Answer from the drawing. Dimensions are ordinates in mm from the lowest x, y and z of the part. A direction names the side the tool comes from. Coordinates: 2 decimals unless noted, no trailing zeros. Write each loop counter-clockwise with the first axis right and the second up, starting at its lowest first coordinate (ties: lowest second). Pieces come first, ordered by that corner, then holes. Notation, with made-up numbers: (46.25, 43.25) -> (86.25, 43.25) arc R18 cw to (86.25, 47.25) -> close; hole circle Ø9 at (59.25, 38). An arc over 180 degrees is marked (long way). One line per item, written item: value. Start each with the question number.
1. Find section C-C, the plane y = 10. Write down the section's boundary in (x, z), and give its area (3 significant figures).
2. For the marked faces 5 and 6, determine the directions among +Z, -Z, +X, -X, +Y, -Y from which every point of the face is accessible in a straight line to the end or side of a thin tool.
3. For a pull along X with two mould halves and no side action, classify the marked faces 1, 2, 3 and 4 as pulls with the +X half, pulls with the -X half, needs draft (parallel to the pull), parting line crosses it, or undercut.
4. Find section B-B, the plane x = 50. Write down the section's boundary in (y, z).
5. Given P1, Ø11, axis at x = 47.5, y = 7.5, coming from the -Z side; P2, Ø6.5, axis at x = 50, y = 10, coming from the -Z side, each flat-ended and moving along its own axis, determine where each tip first touches the part or whether it passes through.
6. Find section A-A, the plane z = 1.25. Write down the section's boundary in (x, y).
7. Find section D-D, the plane z = 10.25. Write down the section's boundary in (x, y), and give its area (3 significant figures).
8. Consider line 1 along Y through (x, z) = (50, 4.4); line 2 along Y through (x, z) = (50, 8); line 3 along X through (y, z) = (25.5, 7.25) (1 decimal). Determine where each line is inside the solid, lowest interval first.
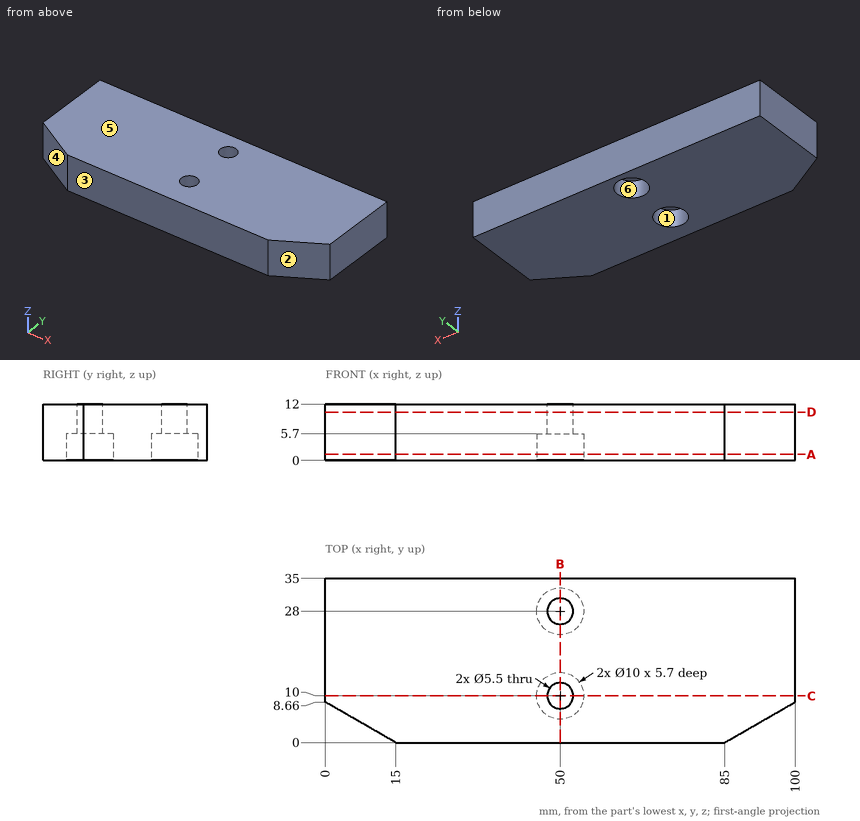
Answer block:
1. outline: (0, 0) -> (45, 0) -> (45, 5.7) -> (47.25, 5.7) -> (47.25, 12) -> (0, 12) -> close; (52.75, 5.7) -> (55, 5.7) -> (55, 0) -> (100, 0) -> (100, 12) -> (52.75, 12) -> close
1. area: 1,110 mm2
2. face 5: +Z, +X, -X, +Y, -Y
2. face 6: -Z
3. face 1: undercut
3. face 2: pulls with the +X half
3. face 3: needs draft
3. face 4: pulls with the -X half
4. outline: (0, 0) -> (5, 0) -> (5, 5.7) -> (7.25, 5.7) -> (7.25, 12) -> (0, 12) -> close; (12.75, 5.7) -> (15, 5.7) -> (15, 0) -> (23, 0) -> (23, 5.7) -> (25.25, 5.7) -> (25.25, 12) -> (12.75, 12) -> close; (30.75, 5.7) -> (33, 5.7) -> (33, 0) -> (35, 0) -> (35, 12) -> (30.75, 12) -> close
5. P1: stops at z = 0
5. P2: stops at z = 5.7
6. outline: (0, 8.66) -> (15, 0) -> (85, 0) -> (100, 8.66) -> (100, 35) -> (0, 35) -> close; hole circle Ø10 at (50, 10); hole circle Ø10 at (50, 28)
7. outline: (0, 8.66) -> (15, 0) -> (85, 0) -> (100, 8.66) -> (100, 35) -> (0, 35) -> close; hole circle Ø5.5 at (50, 10); hole circle Ø5.5 at (50, 28)
7. area: 3,320 mm2
8. line 1: y = 0 to 5, 15 to 23, 33 to 35
8. line 2: y = 0 to 7.25, 12.75 to 25.25, 30.75 to 35
8. line 3: x = 0 to 48.9, 51.1 to 100
